```python
from build123d import *

# Parameters (mm, degrees)
SKETCH_1_W               = 31.6
SKETCH_1_H               = 5
EXTRUDE_1_DEPTH          = 25.8
EXTRUDE_2_DEPTH          = 2
FILLET_1_R               = 4.8
CUT_EXTRUDE_1_DEPTH      = 32.052858162
SKETCH_4_R               = 7.1
CUT_EXTRUDE_2_DEPTH      = 1.5
CHAMFER_2_SIZE           = 0.5
HOLE_WIZARD_1_AT_2_COUNT = 2
HOLE_WIZARD_1_AT_2_PITCH = 42
HOLE_WIZARD_1_AT_3_COUNT = 2
HOLE_WIZARD_1_AT_3_PITCH = 47.413078365
HOLE_WIZARD_1_AT_4_COUNT = 2
HOLE_WIZARD_1_AT_4_PITCH = 22


with BuildPart() as part:
    # 草图1 → 凸台-拉伸1 (new, symmetric)
    with BuildSketch(Plane(origin=(0, 0, 0), x_dir=(0, 0, -1), z_dir=(1, 0, 0))):
        with Locations((0, -2.5)):
            Rectangle(SKETCH_1_W, SKETCH_1_H)
    extrude(amount=EXTRUDE_1_DEPTH, both=True)

    # 草图2 → 凸台-拉伸2 (add)
    with BuildSketch(Plane(origin=(0, 0, 0), x_dir=(1, 0, 0), z_dir=(0, 1, 0))):
        with BuildLine():
            Line((-19.2, 4.5), (-19.2, -4.5))
            ThreePointArc((-19.2, -4.5), (-17.823401872, -7.823401872), (-14.5, -9.2))
            Line((-14.5, -9.2), (14.5, -9.2))
            ThreePointArc((14.5, -9.2), (17.823401872, -7.823401872), (19.2, -4.5))
            Line((19.2, -4.5), (19.2, 4.5))
            ThreePointArc((19.2, 4.5), (17.823401872, 7.823401872), (14.5, 9.2))
            Line((14.5, 9.2), (-14.5, 9.2))
            ThreePointArc((-14.5, 9.2), (-17.823401872, 7.823401872), (-19.2, 4.5))
        make_face()
    extrude(amount=EXTRUDE_2_DEPTH)

    # 圆角1
    fillet_1_edges = [part.edges().sort_by_distance(p)[0] for p in [
        (25.8, -2.5, 15.8),
        (25.8, -2.5, -15.8),
        (-25.8, -2.5, 15.8),
        (-25.8, -2.5, -15.8),
    ]]
    fillet(fillet_1_edges, radius=FILLET_1_R)

    # 草图3 → 切除-拉伸1 (cut, through all)
    with BuildSketch(Plane.XZ.offset(5)):
        with BuildLine():
            Line((-15.3, -3.019933774), (-15.3, 3.019933774))
            ThreePointArc((-15.3, 3.019933774), (-10, 6.1), (-4.7, 3.019933774))
            Line((-4.7, 3.019933774), (-4.7, -3.019933774))
            ThreePointArc((-4.7, -3.019933774), (-10, -6.1), (-15.3, -3.019933774))
        make_face()
        with BuildLine():
            Line((15.3, 3.019933774), (15.3, -3.019933774))
            ThreePointArc((15.3, -3.019933774), (10, -6.1), (4.7, -3.019933774))
            Line((4.7, -3.019933774), (4.7, 3.019933774))
            ThreePointArc((4.7, 3.019933774), (10, 6.1), (15.3, 3.019933774))
        make_face()
    extrude(amount=-CUT_EXTRUDE_1_DEPTH, mode=Mode.SUBTRACT)

    # 草图4 → 切除-拉伸2 (cut)
    with BuildSketch(Plane.XZ.offset(5)):
        with Locations(Location((-10, 0, 0), (0, 0, 270))):
            Circle(SKETCH_4_R)
        with Locations(Location((10, 0, 0), (0, 0, 270))):
            Circle(SKETCH_4_R)
    extrude(amount=-CUT_EXTRUDE_2_DEPTH, mode=Mode.SUBTRACT)

    # 倒角2
    chamfer_2_edges = [part.edges().sort_by_distance(p)[0] for p in [
        (17.823401872, 2, -7.823401872),
        (0, 2, -9.2),
        (-17.823401872, 2, -7.823401872),
        (-19.2, 2, 0),
        (-17.823401872, 2, 7.823401872),
        (0, 2, 9.2),
        (17.823401872, 2, 7.823401872),
        (19.2, 2, 0),
        (25.8, 0, 0),
        (-25.8, 0, 0),
        (0, 0, 15.8),
        (0, 0, -15.8),
        (-24.39411255, 0, 14.39411255),
        (-24.39411255, 0, -14.39411255),
        (24.39411255, 0, 14.39411255),
        (24.39411255, 0, -14.39411255),
    ]]
    chamfer(chamfer_2_edges, length=CHAMFER_2_SIZE)

    # 草图6 → 打孔尺寸(%根据十字)槽半沉头木螺钉的类型1 (revolve, cut)
    with BuildSketch(Plane(origin=(-21, -5, 11), x_dir=(0, 0, -1), z_dir=(1, 0, 0))):
        Polygon((0, 0), (0, 6.16137699), (1.6, 5.2), (1.6, 2.1), (3, 0.7), (3, 0), align=None)
    hole_wizard_1 = revolve(axis=Axis((-21, -11.35, 11), (0, 1, 0)), mode=Mode.SUBTRACT)

    # 打孔尺寸(%根据十字)槽半沉头木螺钉的类型1 at 2: 打孔尺寸(%根据十字)槽半沉头木螺钉的类型1 ×2
    with Locations(*[(i * HOLE_WIZARD_1_AT_2_PITCH, 0, 0) for i in range(1, HOLE_WIZARD_1_AT_2_COUNT)]):
        add(hole_wizard_1, mode=Mode.SUBTRACT)

    # 打孔尺寸(%根据十字)槽半沉头木螺钉的类型1 at 3: 打孔尺寸(%根据十字)槽半沉头木螺钉的类型1 ×2
    with Locations(*[Vector(0.8858315352801553, 0, -0.4640069946705578) * (i * HOLE_WIZARD_1_AT_3_PITCH) for i in range(1, HOLE_WIZARD_1_AT_3_COUNT)]):
        add(hole_wizard_1, mode=Mode.SUBTRACT)

    # 打孔尺寸(%根据十字)槽半沉头木螺钉的类型1 at 4: 打孔尺寸(%根据十字)槽半沉头木螺钉的类型1 ×2
    with Locations(*[(0, 0, -i * HOLE_WIZARD_1_AT_4_PITCH) for i in range(1, HOLE_WIZARD_1_AT_4_COUNT)]):
        add(hole_wizard_1, mode=Mode.SUBTRACT)


solid = part.part
```
Here's how the part is built. I have some questions about the finished solid (model axes, mm). A direction names the side the tool comes from. Give positions to 0.01 mm unless a question says otherwise; leave off trailing zeros. Loops run counter-clockwise (first coordinate to the right, second up) from the corner with the lowest first, then second, coordinate; pieces in that order, holes last. Notation, with made-up numbers: M 2.5,5.5 L 19.5,5.5 A27 cw 19.5,43.5 Z; hole C 70,49.25 d11. An arc over 180 degrees is marked long. Use one line per item in the form item = value. Start each with the question number.
Q1. Will these pins go through, and if not, where does the flat tip stop? pin 1 Ø5 at (x, z) = (21, 11) entering from -Y; pin 2 Ø8 at (x, z) = (-21, -11) entering from +Y; pin 3 Ø3.5 at (x, z) = (-21, -11) entering from -Y; pin 4 Ø2.5 at (x, z) = (21, -11) entering from -Y.
Q2. If we section it at A-A (x = -10): Write out the boundary of the cut face in (y, z).
Q3. If we section it at B-B (z = 0): Write out the boundary of the cut face in (x, y), then the cut area to 3 significant figures.
Q4. Which directions (+Z, -Z, +X, -X, +Y, -Y) give clear straight access to the entire face, cutting with the end or side of a thin tool? Please do faces 1 (the flat face through (4.7, -1, 0)), 2 (the conical face through (-17.532, 1.865, -7.599)), 3 (the cylindrical face through (-17.86, 0.74, 7.787)), 4 (the flat face through (4, -3.5, 0)).
Q5. If we section it at D-D (z = -12): State how many separate pieces and enclosed holes the cut face has, then the cut area to 3 significant figures.
Q6. Thinking about a two-plate mould opening in Z: for faces 5 (the conical face through (-17.599, 1.865, 7.532)), 6 (the cylindrical face through (22.8, -4.7, 13.4)), 7 (the cylindrical face through (17.86, 0.74, -7.787)), which applies, +Z half, -Z half, draft (parallel to the pull), parting line (faces both ways), or undercut?
Q7. I need wall thicknesses on line 1 along Z through (x, y) = (-21, -0.9); line 2 along X through (y, z) = (-4.6, -11); line 3 along X through (y, z) = (-2.2, -11). Which ranges of each line are inside material? Lowest first, please.
Q8. If we section it at C-C (y = -2): Write out the boundary of the cut face in (x, z), then the cut area to 3 significant figures.
Taken from the geometry:
q1.pin_1 = -3.8
q1.pin_2 = 0
q1.pin_3 = -3.05
q1.pin_4 = through
q2.outline = M -5,-15.8 L -0.5,-15.8 L 0,-15.3 L 0,-9.2 L 1.5,-9.2 L 2,-8.7 L 2,-6.1 L -3.5,-6.1 L -3.5,-7.1 L -5,-7.1 Z; M -5,7.1 L -3.5,7.1 L -3.5,6.1 L 2,6.1 L 2,8.7 L 1.5,9.2 L 0,9.2 L 0,15.3 L -0.5,15.8 L -5,15.8 Z
q3.outline = M -25.8,-5 L -17.1,-5 L -17.1,-3.5 L -15.3,-3.5 L -15.3,2 L -18.7,2 L -19.2,1.5 L -19.2,0 L -25.3,0 L -25.8,-0.5 Z; M -4.7,-3.5 L -2.9,-3.5 L -2.9,-5 L 2.9,-5 L 2.9,-3.5 L 4.7,-3.5 L 4.7,2 L -4.7,2 Z; M 15.3,-3.5 L 17.1,-3.5 L 17.1,-5 L 25.8,-5 L 25.8,-0.5 L 25.3,0 L 19.2,0 L 19.2,1.5 L 18.7,2 L 15.3,2 Z
q3.area = 175 mm^2
q4.face_1 = +Y, -Y
q4.face_2 = -Z, -X, +Y
q4.face_3 = +Z, -X, +Y
q4.face_4 = -Y
q5.separate_pieces = 3
q5.enclosed_holes = 0
q5.area = 223 mm^2
q6.face_5 = +Z half
q6.face_6 = undercut
q6.face_7 = -Z half
q7.line_1 = -15.8 to -12.6, -9.4 to 9.4, 12.6 to 15.8
q7.line_2 = -25.8 to -24, -18 to 18, 24 to 25.8
q7.line_3 = -25.8 to -22.6, -19.4 to 19.4, 22.6 to 25.8
q8.outline = M -25.8,-11 A4.8 ccw -21,-15.8 L 21,-15.8 A4.8 ccw 25.8,-11 L 25.8,11 A4.8 ccw 21,15.8 L -21,15.8 A4.8 ccw -25.8,11 Z; hole C -21,-11 d3.2; hole C -21,11 d3.2; hole M -15.3,-3.02 A6.1 ccw -4.7,-3.02 L -4.7,3.02 A6.1 ccw -15.3,3.02 Z; hole M 4.7,-3.02 A6.1 ccw 15.3,-3.02 L 15.3,3.02 A6.1 ccw 4.7,3.02 Z; hole C 21,-11 d3.2; hole C 21,11 d3.2
q8.area = 1,360 mm^2
